Work out the finished part from the listing and answer in its coordinate system (mm). A direction names the side the tool comes from. Give positions to 0.01 mm unless a question says otherwise; leave off trailing zeros. Loops run counter-clockwise (first coordinate to the right, second up) from the corner with the lowest first, then second, coordinate; pieces in that order, holes last. Notation, with made-up numbers: M 0.5,-16.75 L 29.5,-16.75 A21 cw 29.5,-11.75 Z; hole C 33,-34.75 d7. An arc over 180 degrees is marked long. Write item = value, one per line. Start each with the question number.
1. Section C-C on x = 57.5 is taken. Determine the outline of the cut face in (y, z) (3 decimals), plus the area to 3 significant figures.
2. Section B-B on x = 4.5 is taken. Determine the outline of the cut face in (y, z).
3. Flat-ended cylindrical pins translate along their axes: pin 1 Ø3 at (x, y) = (35, -2.5) entering from +Z; pin 2 Ø6 at (x, z) = (41, 3) entering from +Y (3 decimals); pin 3 Ø3 at (x, z) = (34.5, -2.5) entering from -Y. Find the tip coordinate at first contact, or state that the pin passes through.
4. Consider L1, parallel to X at y = 1, z = -5.5; L2, parallel to X at y = 9, z = -6; L3, parallel to Y at x = 19, z = 2.25. Determine where each line is inside the solid, lowest interval first. Write a range as [from, to].
5. For faces 1 (the face through (0, 0, -9)), 2 (the face through (3.76, -7.63, 4.32)), 3 (the face through (35.55, 9.3, -2.06)), determine the directions among +Z, -Z, +X, -X, +Y, -Y from which every point of the face is accessible in a straight line to the end or side of a thin tool.
6. Section A-A on y = 0 is taken. Determine the outline of the cut face in (x, z) (3 decimals).
7. The mould has two halves that part along Z. Classify faces 4 (the face through (7.62, 0, 0)), 5 (the face through (4.93, 0.53, 11.99)), 6 (the face through (10, -9, 5)): released by +Z, released by -Z, zero draft, split by the parting line, or undercut.
```python
from build123d import *

# Parameters (mm, degrees)
SKETCH1_R          = 12
BASE_EXTRUDE_DEPTH = 10
CHAMFER_2_SIZE     = 1.6
FILLET_2_R         = 0.6
CUT_EXTRUDE1_DEPTH = 7.62


with BuildPart() as part:
    # Sketch1 → Base-Extrude (new body)
    with BuildSketch(Plane(origin=(0, 0, 0), x_dir=(0, 0, -1), z_dir=(1, 0, 0))):
        Circle(SKETCH1_R)
    extrude(amount=BASE_EXTRUDE_DEPTH)

    # Sketch2 → Boss-Revolve1 (revolve)
    with BuildSketch(Plane.XY, mode=Mode.PRIVATE) as boss_revolve1_sk:
        Polygon((0, 0), (62.8, 0), (62.8, 6.268), (62.8, 9.525), (27.8072, 9.525), (0, 9.525), align=None)
    revolve(boss_revolve1_sk.sketch.rotate(Axis((0, 0, 0), (1, 0, 0)), 90), axis=Axis((0, 0, 0), (1, 0, 0)))

    # Chamfer 2
    chamfer_2_edges = [part.edges().sort_by_distance(p)[0] for p in [
        (62.8, 0, -9.525),
    ]]
    chamfer(chamfer_2_edges, length=CHAMFER_2_SIZE)

    # Fillet 2
    fillet_2_edges = [part.edges().sort_by_distance(p)[0] for p in [
        (10, 0, -9.525),
    ]]
    fillet(fillet_2_edges, radius=FILLET_2_R)

    # Sketch7 → Cut-Extrude1 (cut)
    with BuildSketch(Plane.ZY):
        Polygon((-8.76789552, 5.062146839), (-8.76789552, -5.062146839), (0, -10.124293677), (8.76789552, -5.062146839), (8.76789552, 5.062146839), (0, 10.124293677), align=None)
    extrude(amount=-CUT_EXTRUDE1_DEPTH, mode=Mode.SUBTRACT)


solid = part.part
```
Verdict:
q1.outline = C 0,0 d19.05
q1.area = 285 mm2
q2.outline = C 0,0 d24; hole M -10.12,0 L -5.06,-8.77 L 5.06,-8.77 L 10.12,0 L 5.06,8.77 L -5.06,8.77 Z
q3.pin_1 = 9.47
q3.pin_2 = 9.525
q3.pin_3 = -9.47
q4.L1 = [7.62, 62.8]
q4.L2 = [0, 10]
q4.L3 = [-9.26, 9.26]
q5.face_1 = +Z, -Z, -X, +Y, -Y
q5.face_2 = -X
q5.face_3 = +X
q6.outline = M 0,-12 L 10,-12 L 10,-10.125 A0.6 cw 10.6,-9.525 L 61.2,-9.525 L 62.8,-7.925 L 62.8,7.925 L 61.2,9.525 L 10.6,9.525 A0.6 cw 10,10.125 L 10,12 L 0,12 L 0,8.768 L 7.62,8.768 L 7.62,-8.768 L 0,-8.768 Z
q7.face_4 = undercut
q7.face_5 = split by the parting line
q7.face_6 = zero draft
